```python
from build123d import *

# Parameters (mm, degrees)
SKETCH1_R           = 5
BOSS_EXTRUDE1_DEPTH = 5
CUT_EXTRUDE1_DEPTH  = 2
SKETCH3_R           = 2.5
BOSS_EXTRUDE2_DEPTH = 12
CHAMFER1_SIZE       = 1


with BuildPart() as part:
    # Sketch1 → Boss-Extrude1 (new body)
    with BuildSketch(Plane.XY):
        Circle(SKETCH1_R)
    extrude(amount=BOSS_EXTRUDE1_DEPTH)

    # Sketch2 → Cut-Extrude1 (cut)
    with BuildSketch(Plane.XY.offset(5)):
        Polygon((2.886751346, 0), (1.443375673, 2.5), (-1.443375673, 2.5), (-2.886751346, 0), (-1.443375673, -2.5), (1.443375673, -2.5), align=None)
    extrude(amount=-CUT_EXTRUDE1_DEPTH, mode=Mode.SUBTRACT)

    # Sketch3 → Boss-Extrude2 (add)
    with BuildSketch(Plane(origin=(0, 0, 0), x_dir=(-1, 0, 0), z_dir=(0, 0, -1))):
        Circle(SKETCH3_R)
    extrude(amount=BOSS_EXTRUDE2_DEPTH)

    # Chamfer1
    chamfer1_edges = [part.edges().sort_by_distance(p)[0] for p in [
        (2.5, 0, -12),
    ]]
    chamfer(chamfer1_edges, length=CHAMFER1_SIZE)


solid = part.part
```
Design review of the part built by this model. Coordinates are the model's own, in mm. A direction names the side the tool comes from. Coordinates: 2 decimals unless noted, no trailing zeros. Order: outer loops, then holes, each group sorted by start corner. A loop starts at its lowest first (then second) coordinate and runs counter-clockwise, first axis right, second up. Notation, with made-up numbers: (22, 30) -> (37, 30) arc R30 cw to (37, 58) -> close; hole circle Ø10 at (-31.75, 11.5). An arc over 180 degrees is marked (long way). One line per item, written item: value. Start each with the question number.
Q1. Insertion check: pin 1 Ø6 at (y, z) = (1.5, -9.5) entering from -X; pin 2 Ø2 at (x, z) = (0, -6.5) entering from -Y; pin 3 Ø0.6 at (x, z) = (0.5, 3.5) entering from +Y. Each pin has a flat end and moves straight along its axis. Give the tip position at first contact, or say it passes through.
Q2. Take a section at D-D, the plane z = -6.5. State the section outline as (x, y) points.
Q3. Take a section at B-B, the plane z = 2.75. State the section outline as (x, y) points, then the cut area to 3 significant figures.
Q4. Take a section at C-C, the plane y = -3.75. State the section outline as (x, z) points, then the cut area to 3 significant figures.
Q5. For probe 1 along Z at (x, y) = (-3, 1.75); probe 2 along Y at (x, z) = (-2, -10.75); probe 3 along Y at (x, z) = (-2, 3.5), list the stretches that pass through material, from the lowest coordinate up.
Q6. Mouldability with a two-part tool opening along Y and no side actions: class faces 1 (the flat face through (2, -2, 5)), 2 (the cylindrical face through (-1.08, -4.88, 2.46)), 3 (the flat face through (-2.175, -1.233, 4.014)) as pulls with the +Y half, pulls with the -Y half, needs draft (parallel to the pull), parting line crosses it, or undercut.
Q7. Take a section at A-A, the plane x = 0. State the section outline as (y, z) points.
Q8. Tool access review of faces 4 (the flat face through (2, -2, 0)), 5 (the flat face through (2.175, 1.233, 4.014)), 6 (the flat face through (0, 0, -12)): name each direction out of +Z, -Z, +X, -X, +Y, -Y from which nothing blocks a thin tool from reaching the whole face with its end or side.
Values follow:
1. pin 1: stops at x = -2.5
1. pin 2: stops at y = -2.5
1. pin 3: stops at y = 5
2. outline: circle Ø5 at (0, 0)
3. outline: circle Ø10 at (0, 0)
3. area: 78.5 mm2
4. outline: (-3.31, 0) -> (3.31, 0) -> (3.31, 5) -> (-3.31, 5) -> close
4. area: 33.1 mm2
5. probe 1: z = 0 to 5
5. probe 2: y = -1.5 to 1.5
5. probe 3: y = -4.58 to -1.54, 1.54 to 4.58
6. face 1: needs draft
6. face 2: parting line crosses it
6. face 3: undercut
7. outline: (-5, 0) -> (-2.5, 0) -> (-2.5, -11) -> (-1.5, -12) -> (1.5, -12) -> (2.5, -11) -> (2.5, 0) -> (5, 0) -> (5, 5) -> (2.5, 5) -> (2.5, 3) -> (-2.5, 3) -> (-2.5, 5) -> (-5, 5) -> close
8. face 4: -Z
8. face 5: +Z
8. face 6: -Z, +X, -X, +Y, -Y
